from build123d import *

# Parameters (mm, degrees)
SKETCH1_W                                            = 40
SKETCH1_H                                            = 10
BOSS_EXTRUDE1_DEPTH                                  = 6
CHAMFER1_SIZE                                        = 0.5
HOLE_SIZE_PER_SOCKET_HEAD_CAP_SCREW_TYPE_D           = 3.4
HOLE_SIZE_PER_SOCKET_HEAD_CAP_SCREW_TYPE_CBORE_D     = 6
HOLE_SIZE_PER_SOCKET_HEAD_CAP_SCREW_TYPE_CBORE_DEPTH = 3.4
SKETCH4_W                                            = 16
SKETCH4_H                                            = 6
CUT_EXTRUDE1_DEPTH                                   = 1
SKETCH5_R                                            = 1.5
CUT_EXTRUDE2_DEPTH                                   = 22.470910554
M3_TAPPED_HOLE1_D                                    = 2.5
M3_TAPPED_HOLE1_DEPTH                                = 5
M3_TAPPED_HOLE1_TIP                                  = 0.751075774


with BuildPart() as part:
    # Sketch1 → Boss-Extrude1 (new body)
    with BuildSketch(Plane.XY):
        Rectangle(SKETCH1_W, SKETCH1_H)
    extrude(amount=BOSS_EXTRUDE1_DEPTH)

    # Chamfer1
    chamfer1_edges = [part.edges().sort_by_distance(p)[0] for p in [
        (-20, 5, 3),
        (20, 5, 3),
        (20, -5, 3),
        (-20, -5, 3),
    ]]
    chamfer(chamfer1_edges, length=CHAMFER1_SIZE)

    # Hole Size per Socket Head Cap Screw Type1 (through all)
    with Locations(Plane.XY.offset(6)):
        with Locations((-14, 0), (14, 0)):
            CounterBoreHole(HOLE_SIZE_PER_SOCKET_HEAD_CAP_SCREW_TYPE_D / 2, HOLE_SIZE_PER_SOCKET_HEAD_CAP_SCREW_TYPE_CBORE_D / 2, HOLE_SIZE_PER_SOCKET_HEAD_CAP_SCREW_TYPE_CBORE_DEPTH)

    # Sketch4 → Cut-Extrude1 (cut)
    with BuildSketch(Plane(origin=(0, -5, 0), x_dir=(1, 0, 0), z_dir=(0, 1, 0))):
        with Locations((0, -3)):
            Rectangle(SKETCH4_W, SKETCH4_H)
    extrude(amount=CUT_EXTRUDE1_DEPTH, mode=Mode.SUBTRACT)

    # Sketch5 → Cut-Extrude2 (cut, through all)
    with BuildSketch(Plane.XY):
        with Locations((-6, 0)):
            Circle(SKETCH5_R)
        with Locations((6, 0)):
            Circle(SKETCH5_R)
    extrude(amount=CUT_EXTRUDE2_DEPTH, mode=Mode.SUBTRACT)

    # M3 Tapped Hole1
    with Locations(Plane(origin=(0, 5, 0), x_dir=(-1, 0, 0), z_dir=(0, 1, 0))):
        with Locations((6, 3), (-6, 3)):
            Hole(M3_TAPPED_HOLE1_D / 2, depth=M3_TAPPED_HOLE1_DEPTH)
            with Locations((0, 0, -(M3_TAPPED_HOLE1_DEPTH + M3_TAPPED_HOLE1_TIP / 2))):  # 118° drill point
                Cone(0, M3_TAPPED_HOLE1_D / 2, M3_TAPPED_HOLE1_TIP, mode=Mode.SUBTRACT)


solid = part.part
Read the model definition and answer for the solid it produces. Units are mm, in the model's axes. A direction names the side the tool comes from. Round coordinates to 2 decimals unless told otherwise and drop trailing zeros. Write each loop counter-clockwise with the first axis right and the second up, starting at its lowest first coordinate (ties: lowest second). Pieces come first, ordered by that corner, then holes.
1. The part is cut by section B-B, the plane x = -14. Determine the outline of the cut face in (y, z).
2. The part is cut by section C-C, the plane x = 6. Determine the outline of the cut face in (y, z).
3. The part is cut by section D-D, the plane z = 2.25. Determine the outline of the cut face in (x, y), then the cut area to 3 significant figures.
4. The part is cut by section A-A, the plane y = 0. Determine the outline of the cut face in (x, z).
5. Straight lines are drawn through the part: L1, parallel to X at y = 1.25, z = 5; L2, parallel to X at y = -1.75, z = 3.5; L3, parallel to X at y = -1, z = 4.75. For each, find the intervals that lie inside material, in ascending order.
6. Given pin 1 Ø3 at (x, z) = (-6, 3) entering from -Y; pin 2 Ø4.5 at (x, y) = (14, 0) entering from +Z; pin 3 Ø5 at (x, y) = (-12.5, -1) entering from +Z; pin 4 Ø2.5 at (x, y) = (-6, 0) entering from +Z, each flat-ended and moving along its own axis, determine where each tip first touches the part or whether it passes through.
7. Which of the six approach directions +Z, -Z, +X, -X, +Y, -Y give full straight-line access (tool end or side, diameter ignored) to faces 1 (the face through (14, -5, 3)), 2 (the face through (-4.81, 2.89, 3.38)), 3 (the face through (0, -4, 3)), 4 (the face through (-12, 0, 2.6)), 5 (the face through (-20, 0, 3))?
8. Determine the mould class of faces 6 (the face through (11, 0, 4)), 7 (the face through (-14, -5, 3)), 8 (the face through (0, 5, 3)) for opening direction Y: pulls with the +Y half, pulls with the -Y half, needs draft (parallel to the pull), parting line crosses it, or undercut.
Values:
1. outline: (-5, 0) - (-1.7, 0) - (-1.7, 2.6) - (-3, 2.6) - (-3, 6) - (-5, 6) - close; (1.7, 0) - (5, 0) - (5, 6) - (3, 6) - (3, 2.6) - (1.7, 2.6) - close
2. outline: (-4, 0) - (-1.5, 0) - (-1.5, 6) - (-4, 6) - close; (1.5, 0) - (5, 0) - (5, 1.75) - (1.5, 1.75) - close; (1.5, 4.25) - (5, 4.25) - (5, 6) - (1.5, 6) - close
3. outline: (-20, -4.5) - (-19.5, -5) - (-8, -5) - (-8, -4) - (8, -4) - (8, -5) - (19.5, -5) - (20, -4.5) - (20, 4.5) - (19.5, 5) - (7, 5) - (7, 1.12) arc R1.5 cw (long way) to (5, 1.12) - (5, 5) - (-5, 5) - (-5, 1.12) arc R1.5 cw (long way) to (-7, 1.12) - (-7, 5) - (-19.5, 5) - (-20, 4.5) - close; hole circle Ø3.4 at (-14, 0); hole circle Ø3.4 at (14, 0)
3. area: 337 mm2
4. outline: (-20, 0) - (-15.7, 0) - (-15.7, 2.6) - (-17, 2.6) - (-17, 6) - (-20, 6) - close; (-12.3, 0) - (-7.5, 0) - (-7.5, 6) - (-11, 6) - (-11, 2.6) - (-12.3, 2.6) - close; (-4.5, 0) - (4.5, 0) - (4.5, 6) - (-4.5, 6) - close; (7.5, 0) - (12.3, 0) - (12.3, 2.6) - (11, 2.6) - (11, 6) - (7.5, 6) - close; (15.7, 0) - (20, 0) - (20, 6) - (17, 6) - (17, 2.6) - (15.7, 2.6) - close
5. L1: x = -20 to -16.73, -11.27 to -6.83, -5.17 to 5.17, 6.83 to 11.27, 16.73 to 20
5. L2: x = -20 to -16.44, -11.56 to 11.56, 16.44 to 20
5. L3: x = -20 to -16.83, -11.17 to -7.12, -4.88 to 4.88, 7.12 to 11.17, 16.83 to 20
6. pin 1: stops at y = -4
6. pin 2: stops at z = 2.6
6. pin 3: stops at z = 6
6. pin 4: passes through
7. face 1: +Z, -Z, +X, -X, -Y
7. face 2: +Y
7. face 3: +Z, -Z, -Y
7. face 4: +Z
7. face 5: +Z, -Z, -X, +Y, -Y
8. face 6: undercut
8. face 7: pulls with the -Y half
8. face 8: pulls with the +Y half
